```python
from build123d import *

# Parameters (mm, degrees)
EXTRUDE_1_DEPTH = 25
EXTRUDE_2_DEPTH = 4
CHAMFER_1_SIZE  = 2


with BuildPart() as part:
    # 草图1 → 凸台-拉伸1 (new, symmetric)
    with BuildSketch(Plane.XY):
        Polygon((0, 0), (217.5, 0), (217.5, 10), (10, 10), (10, 90), (0, 90), align=None)
    extrude(amount=EXTRUDE_1_DEPTH, both=True)

    # 草图2 → 凸台-拉伸2 (add, symmetric)
    with BuildSketch(Plane.XY):
        Polygon((10, 87), (217.5, 20), (217.5, 10), (15, 10), (10, 15), align=None)
    extrude(amount=EXTRUDE_2_DEPTH, both=True)

    # 倒角1
    chamfer_1_edges = [part.edges().sort_by_distance(p)[0] for p in [
        (217.5, 5, 25),
        (5, 90, 25),
        (5, 90, -25),
        (217.5, 5, -25),
    ]]
    chamfer(chamfer_1_edges, length=CHAMFER_1_SIZE)


solid = part.part
```
Could you check a few things on this model? Use its own coordinates, in mm. A direction names the side the tool comes from. Round coordinates to 2 decimals unless told otherwise and drop trailing zeros. Write each loop counter-clockwise with the first axis right and the second up, starting at its lowest first coordinate (ties: lowest second). Pieces come first, ordered by that corner, then holes. Notation, with made-up numbers: M -10,-32.5 L 5,-32.5 A26 cw 5,-6.5 Z; hole C 4,38 d2. An arc over 180 degrees is marked long. Answer in a Markdown table with one row per item. Add a question column.
Q1. If I drill on line 1 (X direction, y = 11.5, z = -19); line 2 (Z direction, x = 205.5, y = 15), over which ranges is the centre line in solid material (lowest first)? Write a range as from..to.
Q2. Will these pins go through, and if not, where does the flat tip stop? pin 1 Ø1.5 at (x, z) = (97, 15.5) entering from +Y; pin 2 Ø1 at (x, y) = (92, 13) entering from +Z; pin 3 Ø15 at (x, z) = (124, -10) entering from +Y.
Q3. Imagine slicing it at C-C (y = 33). Please give me the cut outline in (x, z), then the cut area to 3 significant figures.
Q4. Imagine slicing it at B-B (x = 24). Please give me the cut outline in (y, z).
Q5. On a 3-axis mill with a long thin cutter (end or side, diameter ignored), from which of +Z, -Z, +X, -X, +Y, -Y can I reach the whole of each face in a straight line? I mean faces 1 (the flat face through (92, 40, 4)), 2 (the flat face through (92, 40, -4)), 3 (the flat face through (112.3, 53.97, 0.06)). Say none if no direction works.
Q6. Imagine slicing it at A-A (z = -8). Please give me the cut outline in (x, y), then the cut area to 4 significant figures.
Q7. If we mould it in two halves opening along X, with no side actions, what happens to faces 4 (the flat face through (13, 12, 0)), 5 (the flat face through (0, 46, 0)), 6 (the flat face through (5, 90, 0))? For each: +X half, -X half, draft (parallel to the pull), parting line (faces both ways), or undercut.
Values:
| question | item | result |
|---|---|---|
| 1 | line 1 | 0..10 |
| 1 | line 2 | -4..4 |
| 2 | pin 1 | y = 10 |
| 2 | pin 2 | z = 4 |
| 2 | pin 3 | y = 51.64 |
| 3 | outline | M 0,-25 L 10,-25 L 10,-4 L 177.24,-4 L 177.24,4 L 10,4 L 10,25 L 0,25 Z |
| 3 | area | 1,840 mm^2 |
| 4 | outline | M 0,-25 L 10,-25 L 10,-4 L 82.48,-4 L 82.48,4 L 10,4 L 10,25 L 0,25 Z |
| 5 | face 1 | +Z, +X, +Y |
| 5 | face 2 | -Z, +X, +Y |
| 5 | face 3 | +Z, -Z, +X, +Y |
| 6 | outline | M 0,0 L 217.5,0 L 217.5,10 L 10,10 L 10,90 L 0,90 Z |
| 6 | area | 2,975 mm^2 |
| 7 | face 4 | undercut |
| 7 | face 5 | -X half |
| 7 | face 6 | draft |
